Job drawing, mm, ordinate dimensions from the low corner. One solid piece. A direction names the side the tool comes from. Round coordinates to 2 decimals unless told otherwise and drop trailing zeros. Write each loop counter-clockwise with the first axis right and the second up, starting at its lowest first coordinate (ties: lowest second). Pieces come first, ordered by that corner, then holes.
1) Wall check: probe 1 along Y at (x, z) = (25, 271.5); probe 2 along X at (y, z) = (57.5, 276). Give the ranges that are in metal, low to high.
2) Saw through at A-A (y = 48). Write the cut outline in (x, z).
3) Pull direction X, two halves, no side cores. Call the marked faces 1, 2 and 3: +X half, -X half, draft (parallel to the pull), parting line (faces both ways), or undercut.
4) Saw through at B-B (z = 171.5). Write the cut outline in (x, y), plus the area to 3 significant figures.
5) Which spindle directions (+Z, -Z, +X, -X, +Y, -Y) get a long thin tool onto all of the face, cutting with end or side? Do the marked faces 4 and 5. Say none if no direction does.
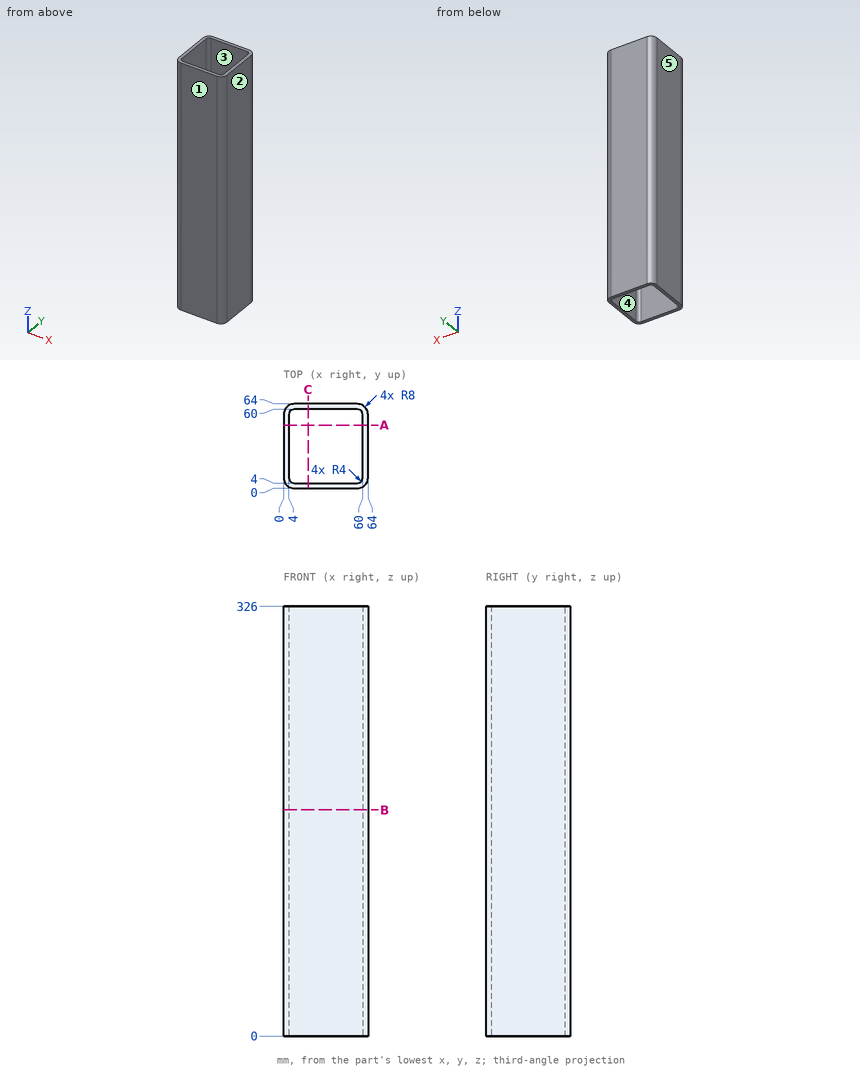
Evaluation:
1. probe 1: y = 0 to 4, 60 to 64
1. probe 2: x = 0.14 to 4.29, 59.71 to 63.86
2. outline: (0, 0) - (4, 0) - (4, 326) - (0, 326) - close; (60, 0) - (64, 0) - (64, 326) - (60, 326) - close
3. face 1: draft
3. face 2: +X half
3. face 3: undercut
4. outline: (0, 8) arc R8 ccw to (8, 0) - (56, 0) arc R8 ccw to (64, 8) - (64, 56) arc R8 ccw to (56, 64) - (8, 64) arc R8 ccw to (0, 56) - close; hole (4, 8) arc R4 ccw to (8, 4) - (56, 4) arc R4 ccw to (60, 8) - (60, 56) arc R4 ccw to (56, 60) - (8, 60) arc R4 ccw to (4, 56) - close
4. area: 919 mm2
5. face 4: +Z, -Z
5. face 5: +Z, -Z, -X, +Y, -Y
